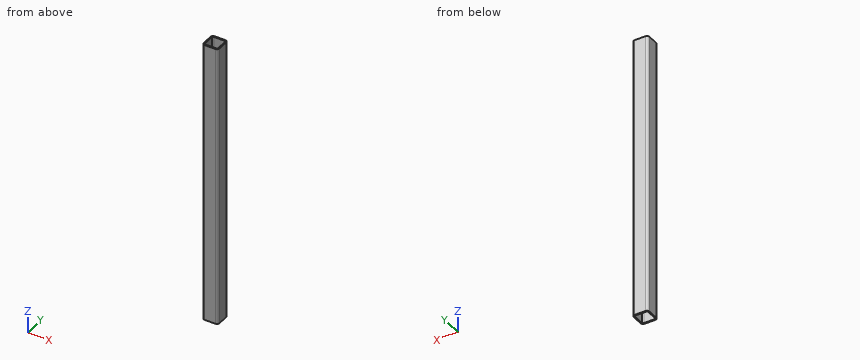
from build123d import *

# Parameters (mm, degrees)
BOSS_EXTRUDE1_DEPTH = 450


with BuildPart() as part:
    # Sketch1 → Boss-Extrude1 (new, symmetric)
    with BuildSketch(Plane.XY):
        with BuildLine():
            Line((-17, -25), (17, -25))
            ThreePointArc((17, -25), (22.656854249, -22.656854249), (25, -17))
            Line((25, -17), (25, 17))
            ThreePointArc((25, 17), (22.656854249, 22.656854249), (17, 25))
            Line((17, 25), (-17, 25))
            ThreePointArc((-17, 25), (-22.656854249, 22.656854249), (-25, 17))
            Line((-25, 17), (-25, -17))
            ThreePointArc((-25, -17), (-22.656854249, -22.656854249), (-17, -25))
        make_face()
        with BuildLine():
            Line((-17, 21), (17, 21))
            ThreePointArc((17, 21), (19.828427125, 19.828427125), (21, 17))
            Line((21, 17), (21, -17))
            ThreePointArc((21, -17), (19.828427125, -19.828427125), (17, -21))
            Line((17, -21), (-17, -21))
            ThreePointArc((-17, -21), (-19.828427125, -19.828427125), (-21, -17))
            Line((-21, -17), (-21, 17))
            ThreePointArc((-21, 17), (-19.828427125, 19.828427125), (-17, 21))
        make_face(mode=Mode.SUBTRACT)
    extrude(amount=BOSS_EXTRUDE1_DEPTH, both=True)


solid = part.part
Verification items for the finished model (mm, model axes). Round coordinates to 2 decimals unless told otherwise and drop trailing zeros. Loops run counter-clockwise (first coordinate to the right, second up) from the corner with the lowest first, then second, coordinate; pieces in that order, holes last. Notation, with made-up numbers: (-9, 64) - (38, 64) arc R10 cw to (38, 82) - close; hole circle Ø2 at (-2, 38). An arc over 180 degrees is marked (long way). Use a Markdown table: item, result. Add a question column.
1. Section check B-B, the plane x = 1. Record the boundary of the cut face in (y, z).
2. Thickness scan on probe 1 along Y at (x, z) = (-13.5, 204); probe 2 along Y at (x, z) = (-20, 85). Record the ranges inside material, lowest first. Write a range as [from, to].
3. Gauge pin test, flat ends, axial feed: pin 1 (2 mm diameter, centred on x = -18, z = 239, fed in from +Y); pin 2 (6 mm diameter, centred on x = 10.5, y = 17.5, fed in from +Z). Record the tip position at first contact, or that the pin passes through.
4. Section check A-A, the plane z = 294. Record the boundary of the cut face in (x, y), plus the area to 3 significant figures.
Checks:
| question | item | result |
|---|---|---|
| 1 | outline | (-25, -450) - (-21, -450) - (-21, 450) - (-25, 450) - close; (21, -450) - (25, -450) - (25, 450) - (21, 450) - close |
| 2 | probe 1 | y = [-25, -21], [21, 25] |
| 2 | probe 2 | y = [-24.42, -19.65], [19.65, 24.42] |
| 3 | pin 1 | stops at y = 25 |
| 3 | pin 2 | passes through |
| 4 | outline | (-25, -17) arc R8 ccw to (-17, -25) - (17, -25) arc R8 ccw to (25, -17) - (25, 17) arc R8 ccw to (17, 25) - (-17, 25) arc R8 ccw to (-25, 17) - close; hole (-21, -17) arc R4 ccw to (-17, -21) - (17, -21) arc R4 ccw to (21, -17) - (21, 17) arc R4 ccw to (17, 21) - (-17, 21) arc R4 ccw to (-21, 17) - close |
| 4 | area | 695 mm^2 |
